from build123d import *

# Parameters (mm, degrees)
BOSS_EXTRUDE1_DEPTH = 554
SKETCH2_W           = 357.128489267
SKETCH2_H           = 514
CUT_EXTRUDE1_DEPTH  = 466
FILLET1_R           = 50
FILLET2_R           = 70
FILLET3_R           = 2


with BuildPart() as part:
    # Sketch1 → Boss-Extrude1 (new body)
    with BuildSketch(Plane.XY):
        with BuildLine():
            Line((0, 0), (0, 150))
            ThreePointArc((0, 150), (-23.431457505, 206.568542495), (-80, 230))
            Line((-80, 230), (-230, 230))
            Line((-230, 230), (-230, 250))
            Line((-230, 250), (-80, 250))
            ThreePointArc((-80, 250), (-9.289321881, 220.710678119), (20, 150))
            Line((20, 150), (20, 0))
            Line((20, 0), (0, 0))
        make_face()
    extrude(amount=BOSS_EXTRUDE1_DEPTH)

    # Sketch2 → Cut-Extrude1 (cut)
    with BuildSketch(Plane(origin=(0, 250, 0), x_dir=(1, 0, 0), z_dir=(0, 1, 0))):
        with Locations((-31.435755366, -277)):
            Rectangle(SKETCH2_W, SKETCH2_H)
    extrude(amount=-CUT_EXTRUDE1_DEPTH, mode=Mode.SUBTRACT)

    # Fillet1
    fillet1_edges = [part.edges().sort_by_distance(p)[0] for p in [
        (-210, 240, 534),
        (-210, 240, 20),
    ]]
    fillet(fillet1_edges, radius=FILLET1_R)

    # Fillet2
    fillet2_edges = [part.edges().sort_by_distance(p)[0] for p in [
        (-230, 240, 554),
        (-230, 240, 0),
    ]]
    fillet(fillet2_edges, radius=FILLET2_R)

    # Fillet3
    fillet3_edges = [part.edges().sort_by_distance(p)[0] for p in [
        (-9.289321881, 220.710678119, 554),
        (20, 75, 0),
        (-120, 250, 554),
        (-23.431457505, 206.568542495, 554),
        (0, 75, 554),
        (0, 75, 534),
        (0, 75, 20),
        (-9.289321881, 220.710678119, 20),
        (20, 75, 20),
        (-23.431457505, 206.568542495, 20),
        (-120, 230, 20),
        (20, 75, 534),
        (-9.289321881, 220.710678119, 534),
        (-23.431457505, 206.568542495, 534),
        (10, 0, 534),
        (10, 0, 554),
        (-120, 250, 20),
        (-210, 250, 277),
        (-210, 230, 277),
        (-120, 230, 534),
        (-120, 250, 534),
        (-195.355339059, 250, 34.644660941),
        (-195.355339059, 230, 34.644660941),
        (-195.355339059, 250, 519.355339059),
        (-195.355339059, 230, 519.355339059),
        (-230, 230, 277),
        (-230, 250, 277),
        (20, 75, 554),
        (-120, 230, 554),
        (-120, 230, 0),
        (-209.497474683, 230, 533.497474683),
        (-209.497474683, 230, 20.502525317),
        (-209.497474683, 250, 533.497474683),
        (-209.497474683, 250, 20.502525317),
        (0, 75, 0),
        (-23.431457505, 206.568542495, 0),
        (-120, 250, 0),
        (-9.289321881, 220.710678119, 0),
    ]]
    fillet(fillet3_edges, radius=FILLET3_R)


solid = part.part
Could you check a few things on this model? Use its own coordinates, in mm. A direction names the side the tool comes from. Round coordinates to 2 decimals unless told otherwise and drop trailing zeros. Loops run counter-clockwise (first coordinate to the right, second up) from the corner with the lowest first, then second, coordinate; pieces in that order, holes last. Notation, with made-up numbers: (63, 43.25) -> (90, 43.25) arc R20 cw to (90, 47.25) -> close; hole circle Ø4 at (56.5, -30). An arc over 180 degrees is marked (long way). Use CSV: the item, a comma, the result in double quotes.
(1) Suppose I cut it at B-B on y = 34. Write out the boundary of the cut face in (x, z).
Return value:
outline,"(0, 2) arc R2 ccw to (2, 0) -> (18, 0) arc R2 ccw to (20, 2) -> (20, 18) arc R2 ccw to (18, 20) -> (2, 20) arc R2 ccw to (0, 18) -> close; (0, 536) arc R2 ccw to (2, 534) -> (18, 534) arc R2 ccw to (20, 536) -> (20, 552) arc R2 ccw to (18, 554) -> (2, 554) arc R2 ccw to (0, 552) -> close"
(2) Suppose I cut it at C-C on z = 226. Write out the boundary of the cut face in (x, y).
Return value:
outline,"(-230, 232) arc R2 ccw to (-228, 230) -> (-212, 230) arc R2 ccw to (-210, 232) -> (-210, 248) arc R2 ccw to (-212, 250) -> (-228, 250) arc R2 ccw to (-230, 248) -> close"
(3) For faces 1 (the flat face through (0, 74, 544)), 2 (the cylindrical face through (-208.95, 240.11, 19.96)), 3 (the flat face through (-5, 189, 20)), which set-ups out of +Z, -Z, +X, -X, +Y, -Y let a thin tool reach every point of the face, with its end or its side?
Return value:
face 1,"+Z, -Z, -X, -Y"
face 2,"-Z, -X, +Y, -Y"
face 3,"+X, +Y, -Y"
(4) Suppose I cut it at A-A on x = -108.5. Write out the boundary of the cut face in (y, z).
Return value:
outline,"(230, 2) arc R2 ccw to (232, 0) -> (248, 0) arc R2 ccw to (250, 2) -> (250, 18) arc R2 ccw to (248, 20) -> (232, 20) arc R2 ccw to (230, 18) -> close; (230, 536) arc R2 ccw to (232, 534) -> (248, 534) arc R2 ccw to (250, 536) -> (250, 552) arc R2 ccw to (248, 554) -> (232, 554) arc R2 ccw to (230, 552) -> close"
(5) If I drill on probe 1 along Y at (x, z) = (-212, 493); probe 2 along Z at (x, y) = (-16, 224); probe 3 along X at (y, z) = (236.5, 155), over which ranges is the centre line in solid material (lowest first)? Write a range as [from, to].
Return value:
probe 1,"y = [230, 250]"
probe 2,"z = [0, 20], [534, 554]"
probe 3,"x = [-230, -210]"
(6) Will these pins go through, and if not, where does the flat tip stop? pin 1 Ø8 at (y, z) = (40.5, 548) entering from -X; pin 2 Ø5 at (y, z) = (242, 321.5) entering from +X.
Return value:
pin 1,"stops at x = 0"
pin 2,"stops at x = -210"
(7) If we mould it in two halves opening along Z, with no side actions, what happens to faces 4 (the flat face through (20, 76, 10)), 5 (the flat face through (-210, 240, 280)), 6 (the cylindrical face through (-210.04, 240.11, 532.95))? For each: +Z half, -Z half, draft (parallel to the pull), parting line (faces both ways), or undercut.
Return value:
face 4,"draft"
face 5,"undercut"
face 6,"+Z half"
